```python
from build123d import *

# Parameters (mm, degrees)
SKETCH_1_R      = 18
EXTRUDE_1_DEPTH = 8


with BuildPart() as part:
    # 草图1 → 拉伸1 (new body)
    with BuildSketch(Plane.XY):
        with BuildLine():
            Line((-2.5, 24.871068248), (-2.5, 22))
            Line((-2.5, 22), (2.5, 22))
            Line((2.5, 22), (2.5, 24.871068248))
            ThreePointArc((2.5, 24.871068248), (17.675124268, 17.675124268), (24.871068248, 2.5))
            Line((24.871068248, 2.5), (22, 2.5))
            Line((22, 2.5), (22, -2.5))
            Line((22, -2.5), (24.871068248, -2.5))
            ThreePointArc((24.871068248, -2.5), (17.675124268, -17.675124268), (2.5, -24.871068248))
            Line((2.5, -24.871068248), (2.5, -22))
            Line((2.5, -22), (-2.5, -22))
            Line((-2.5, -22), (-2.5, -24.871068248))
            ThreePointArc((-2.5, -24.871068248), (-17.675124268, -17.675124268), (-24.871068248, -2.5))
            Line((-24.871068248, -2.5), (-22, -2.5))
            Line((-22, -2.5), (-22, 2.5))
            Line((-22, 2.5), (-24.871068248, 2.5))
            ThreePointArc((-24.871068248, 2.5), (-17.675124268, 17.675124268), (-2.5, 24.871068248))
        make_face()
        Circle(SKETCH_1_R, mode=Mode.SUBTRACT)
    extrude(amount=EXTRUDE_1_DEPTH)


solid = part.part
```
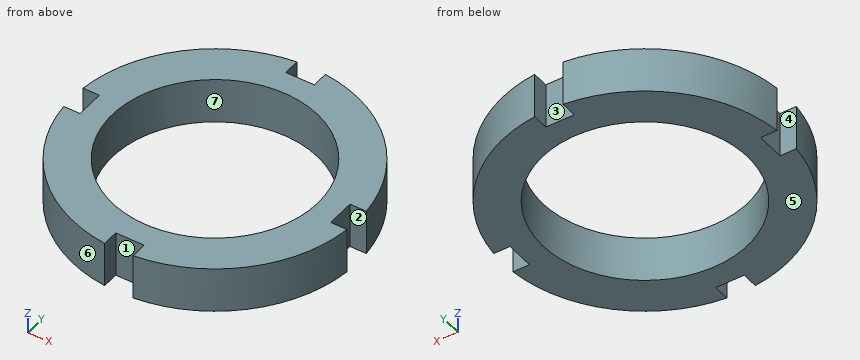
Read the model definition and answer for the solid it produces. Units are mm, in the model's axes. Face numbers are marked on the shaded views. A direction names the side the tool comes from. Coordinates: 2 decimals unless noted, no trailing zeros. Write each loop counter-clockwise with the first axis right and the second up, starting at its lowest first coordinate (ties: lowest second). Pieces come first, ordered by that corner, then holes. Notation, with made-up numbers: (11, 65.5) -> (34, 65.5) arc R14 ccw to (34, 74.5) -> close; hole circle Ø8 at (85.5, 81). An arc over 180 degrees is marked (long way). Return JSON: item names as keys, results as strings.
1. A cutting plane is placed at A-A (x = 0). Determine the outline of the cut face in (y, z).
Found:
{"outline": "(-22, 0) -> (-18, 0) -> (-18, 8) -> (-22, 8) -> close; (18, 0) -> (22, 0) -> (22, 8) -> (18, 8) -> close"}
2. A cutting plane is placed at C-C (z = 2.5). Determine the outline of the cut face in (x, y), and give its area (3 significant figures).
Found:
{"outline": "(-24.87, -2.5) arc R25 ccw to (-2.5, -24.87) -> (-2.5, -22) -> (2.5, -22) -> (2.5, -24.87) arc R25 ccw to (24.87, -2.5) -> (22, -2.5) -> (22, 2.5) -> (24.87, 2.5) arc R25 ccw to (2.5, 24.87) -> (2.5, 22) -> (-2.5, 22) -> (-2.5, 24.87) arc R25 ccw to (-24.87, 2.5) -> (-22, 2.5) -> (-22, -2.5) -> close; hole circle Ø36 at (0, 0)", "area": "886 mm2"}
3. A tool of negligible diameter and unlimited length cuts with its end or side. For the marked faces 1, 2, 3 and 4, from which of +Z, -Z, +X, -X, +Y, -Y can it reach the whole face along a straight path? Write none if from no direction.
Found:
{"face 1": "+Z, -Z, -Y", "face 2": "+Z, -Z, +X", "face 3": "+Z, -Z, +Y", "face 4": "+Z, -Z, -X"}
4. Each of these flat-tipped pins is pushed along its axis until it touches: P1, Ø1.4, axis at y = -23.5, z = 5.5, coming from the +X side; P2, Ø3, axis at x = 23.5, z = 3, coming from the -Y side; P3, Ø1.5, axis at y = -0.5, z = 5.5, coming from the -X side. Where does it stop, or does it pass through?
Found:
{"P1": "x = 10.25", "P2": "y = -11.87", "P3": "x = -22"}
5. Determine the mould class of the marked faces 5, 6 and 7 for opening direction Y: pulls with the +Y half, pulls with the -Y half, needs draft (parallel to the pull), parting line crosses it, or undercut.
Found:
{"face 5": "needs draft", "face 6": "pulls with the -Y half", "face 7": "undercut"}
6. Find the intervals of material crossed by line 1 along Y through (x, z) = (0, 3); line 2 along X through (y, z) = (-12.5, 2.5); line 3 along Y through (x, z) = (-23, 1.5), in increasing order. Write a range as from..to.
Found:
{"line 1": "-22..-18, 18..22", "line 2": "-21.65..-12.95, 12.95..21.65", "line 3": "-9.79..-2.5, 2.5..9.79"}
7. A cutting plane is placed at D-D (y = -20). Determine the outline of the cut face in (x, z), and give its area (3 significant figures).
Found:
{"outline": "(-14.99, 0) -> (14.99, 0) -> (14.99, 8) -> (-14.99, 8) -> close", "area": "240 mm2"}
